Geometry check sheet. Reference: drawing and pictorial views, mm from the part's lowest x, y, z. Give positions to 0.01 mm unless a question says otherwise; leave off trailing zeros. Write each loop counter-clockwise with the first axis right and the second up, starting at its lowest first coordinate (ties: lowest second). Pieces come first, ordered by that corner, then holes. Notation, with made-up numbers: (84.25, 52.5) -> (117.25, 52.5) arc R9 ccw to (117.25, 67.5) -> close; hole circle Ø5 at (10.25, -23.5). An arc over 180 degrees is marked (long way). Return JSON: item names as keys, results as strings.
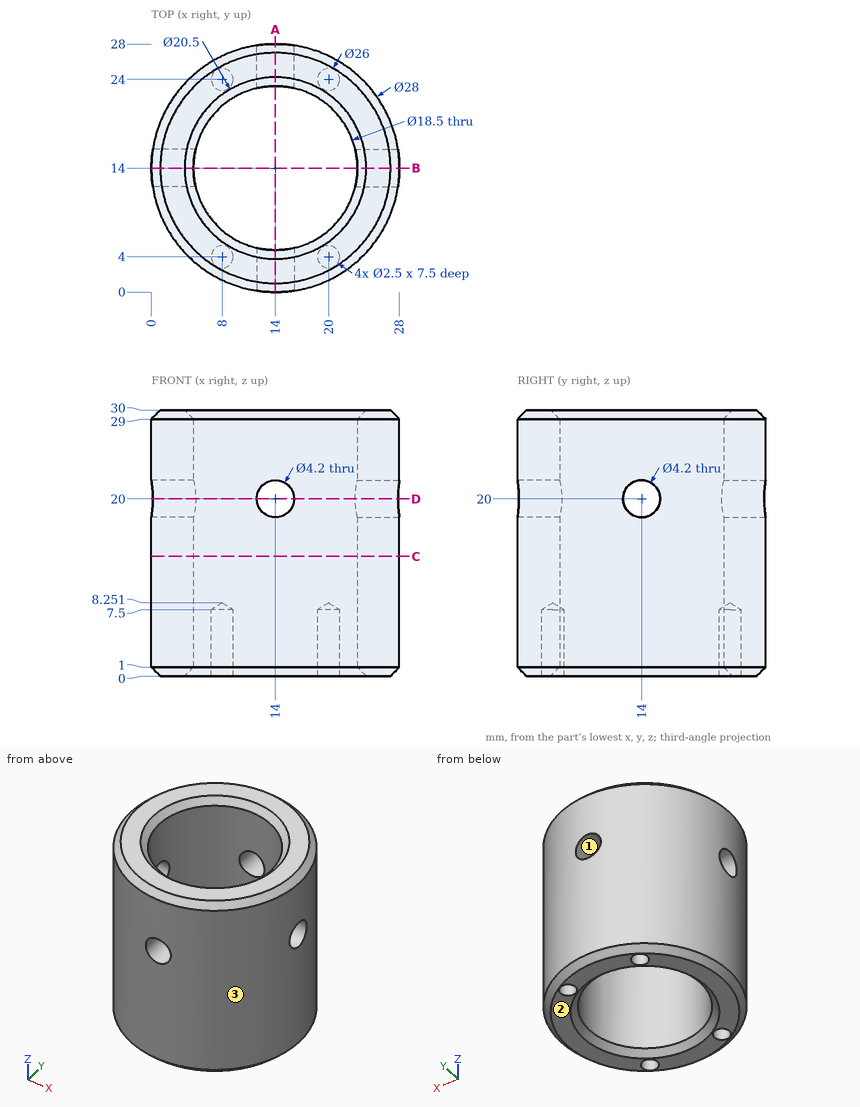
(1) Cross-section at C-C on z = 13.5. Enter the section's corners in (x, y), then the cut area to 3 significant figures.
Reply:
{"outline": "circle Ø28 at (14, 14); hole circle Ø18.5 at (14, 14)", "area": "347 mm^2"}
(2) Depth check by flat-ended pin: pin 1 Ø2 at (x, y) = (20, 24) entering from -Z; pin 2 Ø2 at (x, z) = (24, 16.5) entering from -Y; pin 3 Ø1 at (y, z) = (18.5, 14.5) entering from -X. Enter the tip coordinate at first touch or a pass-through.
Reply:
{"pin 1": "z = 7.65", "pin 2": "y = 3.28", "pin 3": "x = 0.58"}
(3) Thickness scan on L1, parallel to Z at x = 14, y = 26.25; L2, parallel to X at y = 3, z = 6.25; L3, parallel to Y at x = 8, z = 4. Record the ranges inside material, lowest first.
Reply:
{"L1": "0 to 17.9, 22.1 to 30", "L2": "5.34 to 7.25, 8.75 to 19.25, 20.75 to 22.66", "L3": "1.35 to 2.75, 5.25 to 6.96, 21.04 to 22.75, 25.25 to 26.65"}
(4) Release check for a two-part mould opening along X. For the marked faces 1, 2 and 3 record: pulls with the +X half, pulls with the -X half, needs draft (parallel to the pull), parting line crosses it, or undercut.
Reply:
{"face 1": "undercut", "face 2": "needs draft", "face 3": "parting line crosses it"}
(5) Cross-section at A-A on x = 14. Enter the section's corners in (y, z), then the cut area to 3 significant figures.
Reply:
{"outline": "(0, 1) -> (1, 0) -> (3.75, 0) -> (4.75, 1) -> (4.75, 17.9) -> (0, 17.9) -> close; (0, 22.1) -> (4.75, 22.1) -> (4.75, 29) -> (3.75, 30) -> (1, 30) -> (0, 29) -> close; (23.25, 1) -> (24.25, 0) -> (27, 0) -> (28, 1) -> (28, 17.9) -> (23.25, 17.9) -> close; (23.25, 22.1) -> (28, 22.1) -> (28, 29) -> (27, 30) -> (24.25, 30) -> (23.25, 29) -> close", "area": "241 mm^2"}
(6) Cross-section at D-D on z = 20. Enter the section's corners in (x, y).
Reply:
{"outline": "(0.16, 11.9) arc R14 ccw to (11.9, 0.16) -> (11.9, 4.99) arc R9.25 cw to (4.99, 11.9) -> close; (0.16, 16.1) -> (4.99, 16.1) arc R9.25 cw to (11.9, 23.01) -> (11.9, 27.84) arc R14 ccw to start; (16.1, 0.16) arc R14 ccw to (27.84, 11.9) -> (23.01, 11.9) arc R9.25 cw to (16.1, 4.99) -> close; (16.1, 23.01) arc R9.25 cw to (23.01, 16.1) -> (27.84, 16.1) arc R14 ccw to (16.1, 27.84) -> close"}
